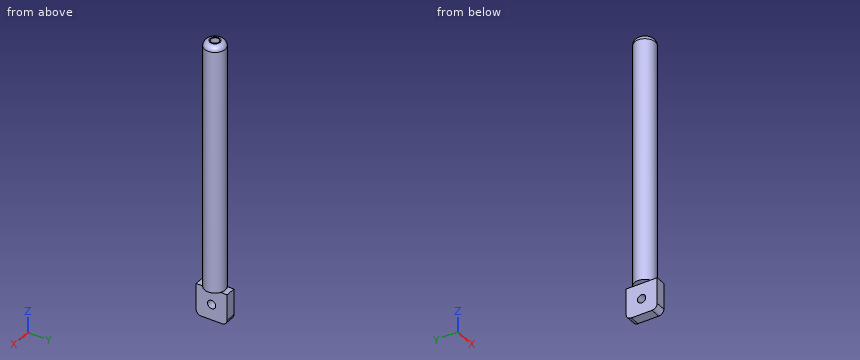
```python
from build123d import *

# Parameters (mm, degrees)
SKETCH1_R           = 10
BOSS_EXTRUDE1_DEPTH = 240
SKETCH2_W           = 30
SKETCH2_H           = 30
BOSS_EXTRUDE2_DEPTH = 5
SKETCH3_R           = 4
CUT_EXTRUDE1_DEPTH  = 38
FILLET1_R           = 5
FILLET2_R           = 5
SKETCH4_R           = 4
CUT_EXTRUDE2_DEPTH  = 20


with BuildPart() as part:
    # Sketch1 → Boss-Extrude1 (new body)
    with BuildSketch(Plane.XY):
        Circle(SKETCH1_R)
    extrude(amount=BOSS_EXTRUDE1_DEPTH)

    # Sketch2 → Boss-Extrude2 (add, symmetric)
    with BuildSketch(Plane(origin=(0, 0, 0), x_dir=(0, 0, -1), z_dir=(1, 0, 0))):
        with Locations((15, 0)):
            Rectangle(SKETCH2_W, SKETCH2_H)
    extrude(amount=BOSS_EXTRUDE2_DEPTH, both=True)

    # Sketch3 → Cut-Extrude1 (cut)
    with BuildSketch(Plane(origin=(5, 0, 0), x_dir=(0, 0, -1), z_dir=(1, 0, 0))):
        with Locations((15, 0)):
            Circle(SKETCH3_R)
    extrude(amount=-CUT_EXTRUDE1_DEPTH, mode=Mode.SUBTRACT)

    # Fillet1
    fillet1_edges = [part.edges().sort_by_distance(p)[0] for p in [
        (0, -15, -30),
        (0, 15, -30),
    ]]
    fillet(fillet1_edges, radius=FILLET1_R)

    # Fillet2
    fillet2_edges = [part.edges().sort_by_distance(p)[0] for p in [
        (-10, 0, 240),
    ]]
    fillet(fillet2_edges, radius=FILLET2_R)

    # Sketch4 → Cut-Extrude2 (cut)
    with BuildSketch(Plane.XY.offset(240)):
        Circle(SKETCH4_R)
    extrude(amount=-CUT_EXTRUDE2_DEPTH, mode=Mode.SUBTRACT)


solid = part.part
```
Source: CAD feature listing. Evaluate the final solid. Frame: model axes, mm. Round coordinates to 2 decimals unless told otherwise and drop trailing zeros. Loops run counter-clockwise (first coordinate to the right, second up) from the corner with the lowest first, then second, coordinate; pieces in that order, holes last.
1. Ray query, L1, parallel to Y at x = 2.5, z = -15; L2, parallel to Y at x = 0.5, z = 40; L3, parallel to X at y = -0.75, z = 115.5. Return the intervals inside material, ascending.
2. Section query A-A on z = -15. Output: boundary loops of the cut face in (x, y).
3. Contact query for flat-ended pins moving along their axis: pin 1 (15 mm diameter, centred on y = -5.5, z = -9.5, fed in from -X); pin 2 (7 mm diameter, centred on y = 0, z = -15, fed in from -X); pin 3 (5 mm diameter, centred on x = 0, y = 0, fed in from +Z); pin 4 (5 mm diameter, centred on x = 0.5, z = 130, fed in from +Y). Output: stop coordinate, or through.
Answers below:
1. L1: y = -15 to -4, 4 to 15
1. L2: y = -9.99 to 9.99
1. L3: x = -9.97 to 9.97
2. outline: (-5, -15) - (5, -15) - (5, -4) - (-5, -4) - close; (-5, 4) - (5, 4) - (5, 15) - (-5, 15) - close
3. pin 1: stops at x = -5
3. pin 2: passes through
3. pin 3: stops at z = 220
3. pin 4: stops at y = 10
